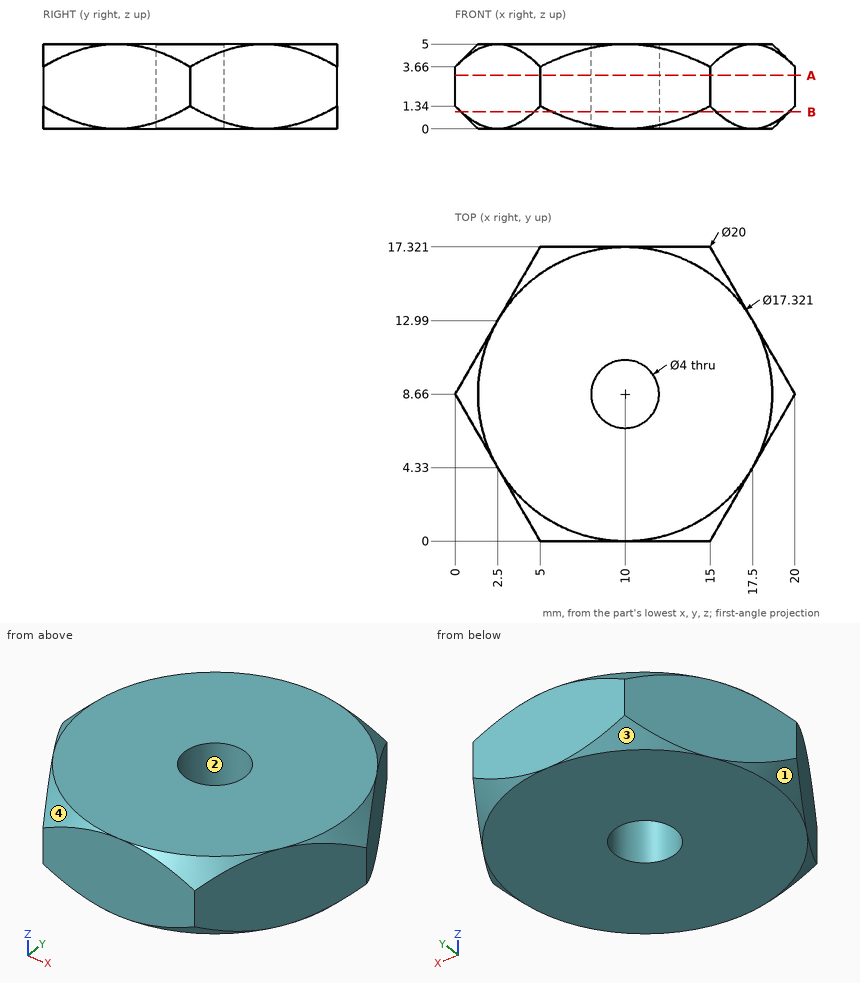
Can you work these out from the drawing? Everything is in mm from the part's minimum corner. Coordinates: 2 decimals unless noted, no trailing zeros. Loops run counter-clockwise (first coordinate to the right, second up) from the corner with the lowest first, then second, coordinate; pieces in that order, holes last. Notation, with made-up numbers: (30.25, 54) - (53.25, 54) arc R21 cw to (53.25, 74) - close; hole circle Ø1 at (26, 48). An arc over 180 degrees is marked (long way). Use a Markdown table: item, result.
Item 1: We'd pull the mould along Y, two halves only. Please class the marked faces 1, 2, 3 and 4: released by +Y, released by -Y, zero draft, split by the parting line, or undercut.
Numbers:
| item | result |
|---|---|
| face 1 | split by the parting line |
| face 2 | undercut |
| face 3 | released by +Y |
| face 4 | released by -Y |
Item 2: If I drill on probe 1 along Y at (x, z) = (10, 2.45); probe 2 along X at (y, z) = (7.75, 4) (1 decimal); probe 3 along Y at (x, z) = (8.25, 1.7) (1 decimal), over which ranges is the centre line in solid material (lowest first)? Write a range as from..to.
Numbers:
| item | result |
|---|---|
| probe 1 | y = 0..6.66, 10.66..17.32 |
| probe 2 | x = 0.5..8.2, 11.8..19.5 |
| probe 3 | y = 0..7.7, 9.6..17.3 |
Item 3: I want a section at B-B on z = 1. Please give me the cut outline in (x, y).
Numbers:
| item | result |
|---|---|
| outline | (0.36, 8.04) - (4.64, 0.62) arc R9.66 ccw to (5.72, 0) - (14.28, 0) arc R9.66 ccw to (15.36, 0.62) - (19.64, 8.04) arc R9.66 ccw to (19.64, 9.28) - (15.36, 16.7) arc R9.66 ccw to (14.28, 17.32) - (5.72, 17.32) arc R9.66 ccw to (4.64, 16.7) - (0.36, 9.28) arc R9.66 ccw to start; hole circle Ø4 at (10, 8.66) |
Item 4: I want a section at A-A on z = 3.15. Please give me the cut outline in (x, y), and give its area (3 significant figures).
Numbers:
| item | result |
|---|---|
| outline | (0, 8.66) - (5, 0) - (15, 0) - (20, 8.66) - (15, 17.32) - (5, 17.32) - close; hole circle Ø4 at (10, 8.66) |
| area | 247 mm2 |
Item 5: Will these pins go through, and if not, where does the flat tip stop? pin 1 (3 mm diameter, centred on y = 12, z = 1, fed in from +X); pin 2 (1.5 mm diameter, centred on x = 15.5, z = 1, fed in from -Y).
Numbers:
| item | result |
|---|---|
| pin 1 | stops at x = 18.94 |
| pin 2 | stops at y = 0 |
